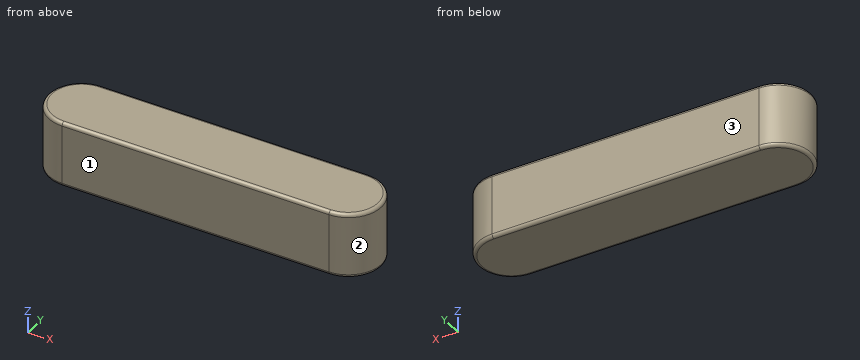
from build123d import *

# Parameters (mm, degrees)
BASE_EXTRUDE_DEPTH = 5
FILLET1_R          = 0.25


with BuildPart() as part:
    # Sketch1 → Base-Extrude (new body)
    with BuildSketch(Plane.XY):
        with BuildLine():
            Line((-10, 2.5), (10, 2.5))
            ThreePointArc((10, 2.5), (12.5, 0), (10, -2.5))
            Line((10, -2.5), (-10, -2.5))
            ThreePointArc((-10, -2.5), (-12.5, 0), (-10, 2.5))
        make_face()
    extrude(amount=BASE_EXTRUDE_DEPTH)

    # Fillet1
    fillet1_edges = [part.edges().sort_by_distance(p)[0] for p in [
        (12.5, 0, 5),
        (0, 2.5, 5),
        (-12.5, 0, 5),
        (0, 2.5, 0),
        (12.5, 0, 0),
        (0, -2.5, 0),
        (-12.5, 0, 0),
        (0, -2.5, 5),
    ]]
    fillet(fillet1_edges, radius=FILLET1_R)


solid = part.part
For this review, take the finished solid that the model builds, in its own axes (mm). Face numbers are marked on the shaded views. Round coordinates to 2 decimals unless told otherwise and drop trailing zeros. Order: outer loops, then holes, each group sorted by start corner. A loop starts at its lowest first (then second) coordinate and runs counter-clockwise, first axis right, second up. Notation, with made-up numbers: M 36.25,-7.5 L 59.25,-7.5 A12 cw 59.25,-0.5 Z; hole C -24,71 d1. An arc over 180 degrees is marked long. Use a Markdown table: item, result. Add a question column.
Item 1: Add section A-A, the plane z = 4.35. Give the boundary of the cut face in (x, y).
Item 2: Mouldability with a two-part tool opening along Y and no side actions: class the marked faces 1, 2 and 3 as released by +Y, released by -Y, zero draft, split by the parting line, or undercut.
Item 3: To check wall thickness, follow line 1 along X through (y, z) = (-1.45, 1.4); line 2 along X through (y, z) = (-0.5, 3.2); line 3 along Y through (x, z) = (-11, 3). State the ranges of each line that lie inside material, in increasing order.
Geometry results:
| question | item | result |
|---|---|---|
| 1 | outline | M -10,-2.5 L 10,-2.5 A2.5 ccw 10,2.5 L -10,2.5 A2.5 ccw Z |
| 2 | face 1 | released by -Y |
| 2 | face 2 | split by the parting line |
| 2 | face 3 | released by +Y |
| 3 | line 1 | x = -12.04 to 12.04 |
| 3 | line 2 | x = -12.45 to 12.45 |
| 3 | line 3 | y = -2.29 to 2.29 |
